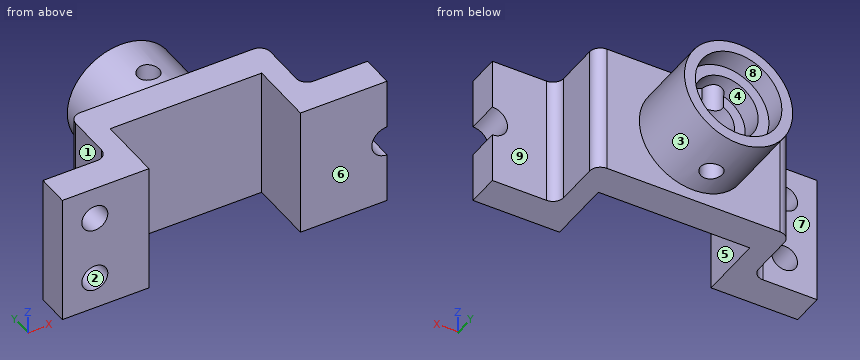
from build123d import *

# Parameters (mm, degrees)
BRACKET_BODY_DEPTH    = 30
FOOT_SLOT_A_REACH     = 88.168
FOOT_SLOT_A_SKETCH_R  = 6
FOOT_SLOT_B_REACH     = 88.168
BEARING_BOSS_SKETCH_R = 25
BEARING_BOSS_DEPTH    = 35
BORE_STEP_1_SKETCH_R  = 20
BORE_STEP_1_DEPTH     = 10
BORE_STEP_2_SKETCH_R  = 15
BORE_STEP_2_DEPTH     = 10
BORE_STEP_3_SKETCH_R  = 10
BORE_STEP_3_DEPTH     = 10
BORE_STEP_4_SKETCH_R  = 5
BORE_STEP_4_DEPTH     = 10
CROSS_HOLE_SKETCH_R   = 5
CROSS_HOLE_DEPTH      = 109.282039139
BEND_FILLET_R5_A_R    = 5
BEND_FILLET_R5_B_R    = 5
BEND_FILLET_R5_C_R    = 5


with BuildPart() as part:
    # Bracket Profile Sketch → Bracket Body (new, symmetric)
    with BuildSketch(Plane.XY):
        Polygon((-75, -30), (-35, -30), (-35, 0), (35, 0), (35, -30), (75, -30), (75, -15), (45, -15), (45, 15), (-45, 15), (-45, -15), (-75, -15), align=None)
    extrude(amount=BRACKET_BODY_DEPTH, both=True)

    # Foot Slot A Sketch → Foot Slot A (cut, up to next)
    with BuildSketch(Plane(origin=(0, -15, 0), x_dir=(1, 0, 0), z_dir=(0, 1, 0)), mode=Mode.PRIVATE) as foot_slot_a_sk1:
        with Locations(Location((-60, 15, 0), (0, 0, 180))):
            Circle(FOOT_SLOT_A_SKETCH_R)
    foot_slot_a_tool1 = extrude(foot_slot_a_sk1.sketch, amount=-FOOT_SLOT_A_REACH, mode=Mode.PRIVATE) & part.part
    # Foot Slot A Sketch → Foot Slot A (cut, up to next)
    with BuildSketch(Plane(origin=(0, -15, 0), x_dir=(1, 0, 0), z_dir=(0, 1, 0)), mode=Mode.PRIVATE) as foot_slot_a_sk2:
        with Locations(Location((-60, -15, 0), (0, 0, 180))):
            Circle(FOOT_SLOT_A_SKETCH_R)
    foot_slot_a_tool2 = extrude(foot_slot_a_sk2.sketch, amount=-FOOT_SLOT_A_REACH, mode=Mode.PRIVATE) & part.part
    add(foot_slot_a_tool1.solids().sort_by_distance((-60, -15, -15))[0], mode=Mode.SUBTRACT)
    add(foot_slot_a_tool2.solids().sort_by_distance((-60, -15, 15))[0], mode=Mode.SUBTRACT)

    # Foot Slot B Sketch → Foot Slot B (cut, up to next)
    with BuildSketch(Plane(origin=(0, -15, 0), x_dir=(1, 0, 0), z_dir=(0, 1, 0)), mode=Mode.PRIVATE) as foot_slot_b_sk1:
        with BuildLine():
            Line((75, 7), (75, -7))
            ThreePointArc((75, -7), (68, 0), (75, 7))
        make_face()
    foot_slot_b_tool1 = extrude(foot_slot_b_sk1.sketch, amount=-FOOT_SLOT_B_REACH, mode=Mode.PRIVATE) & part.part
    add(foot_slot_b_tool1.solids().sort_by_distance((72.029108, -15, 0))[0], mode=Mode.SUBTRACT)

    # Bearing Boss Sketch → Bearing Boss (add)
    with BuildSketch(Plane(origin=(0, 15, 0), x_dir=(1, 0, 0), z_dir=(0, 1, 0))):
        with Locations(Location((0, 0, 0), (0, 0, 180))):
            Circle(BEARING_BOSS_SKETCH_R)
    extrude(amount=BEARING_BOSS_DEPTH)

    # Bore Step 1 Sketch → Bore Step 1 (cut)
    with BuildSketch(Plane(origin=(0, 50, 0), x_dir=(1, 0, 0), z_dir=(0, 1, 0))):
        with Locations(Location((0, 0, 0), (0, 0, 180))):
            Circle(BORE_STEP_1_SKETCH_R)
    extrude(amount=-BORE_STEP_1_DEPTH, mode=Mode.SUBTRACT)

    # Bore Step 2 Sketch → Bore Step 2 (cut)
    with BuildSketch(Plane(origin=(0, 40, 0), x_dir=(1, 0, 0), z_dir=(0, 1, 0))):
        with Locations(Location((0, 0, 0), (0, 0, 180))):
            Circle(BORE_STEP_2_SKETCH_R)
    extrude(amount=-BORE_STEP_2_DEPTH, mode=Mode.SUBTRACT)

    # Bore Step 3 Sketch → Bore Step 3 (cut)
    with BuildSketch(Plane(origin=(0, 30, 0), x_dir=(1, 0, 0), z_dir=(0, 1, 0))):
        with Locations(Location((0, 0, 0), (0, 0, 180))):
            Circle(BORE_STEP_3_SKETCH_R)
    extrude(amount=-BORE_STEP_3_DEPTH, mode=Mode.SUBTRACT)

    # Bore Step 4 Sketch → Bore Step 4 (cut)
    with BuildSketch(Plane(origin=(0, 20, 0), x_dir=(1, 0, 0), z_dir=(0, 1, 0))):
        with Locations(Location((0, 0, 0), (0, 0, 180))):
            Circle(BORE_STEP_4_SKETCH_R)
    extrude(amount=-BORE_STEP_4_DEPTH, mode=Mode.SUBTRACT)

    # Cross Hole Sketch → Cross Hole (cut, through all)
    with BuildSketch(Plane.XY.offset(30)):
        with Locations((0, 29)):
            Circle(CROSS_HOLE_SKETCH_R)
    extrude(amount=-CROSS_HOLE_DEPTH, mode=Mode.SUBTRACT)

    # Bend Fillet R5 A
    bend_fillet_r5_a_edges = [part.edges().sort_by_distance(p)[0] for p in [
        (45, -15, 0),
    ]]
    fillet(bend_fillet_r5_a_edges, radius=BEND_FILLET_R5_A_R)

    # Bend Fillet R5 B
    bend_fillet_r5_b_edges = [part.edges().sort_by_distance(p)[0] for p in [
        (-45, 15, 0),
        (45, 15, 0),
    ]]
    fillet(bend_fillet_r5_b_edges, radius=BEND_FILLET_R5_B_R)

    # Bend Fillet R5 C
    bend_fillet_r5_c_edges = [part.edges().sort_by_distance(p)[0] for p in [
        (-45, -15, 0),
    ]]
    fillet(bend_fillet_r5_c_edges, radius=BEND_FILLET_R5_C_R)


solid = part.part
Design review of the part built by this model. Coordinates are the model's own, in mm. Face numbers are marked on the shaded views. A direction names the side the tool comes from. Round coordinates to 2 decimals unless told otherwise and drop trailing zeros. Order: outer loops, then holes, each group sorted by start corner. A loop starts at its lowest first (then second) coordinate and runs counter-clockwise, first axis right, second up. Notation, with made-up numbers: M -13.5,32 L 17.5,32 A16 ccw 17.5,48 Z; hole C -17.75,-1 d8. An arc over 180 degrees is marked long. Answer as CSV lines item,"result". Start each with the question number.
1) For pin 1 Ø3 at (x, z) = (-11, -6.5) entering from +Y; pin 2 Ø12.5 at (x, z) = (-56.5, 13.5) entering from +Y; pin 3 Ø22 at (y, z) = (4, 8.5) entering from +X; pin 4 Ø11 at (x, z) = (-60, -15) entering from -Y, all flat-tipped, find the tip position at first contact; note any pin that passes through.
2) Tool access review of the marked faces 5, 6, 7, 8 and 9: name each direction out of +Z, -Z, +X, -X, +Y, -Y from which nothing blocks a thin tool from reaching the whole face with its end or side.
3) Add section B-B (y = -3). Give the boundary of the cut face in (x, z), then the cut area to 3 significant figures.
4) Wall thickness on line 1 along Z through (x, y) = (-60, -26.75); line 2 along X through (y, z) = (-6.5, 2.5); line 3 along X through (y, z) = (2, 25): over which ranges is each line inside the solid? List them lowest first. Write a range as [from, to].
5) The part is to be moulded in two halves that separate along X. For the marked faces 1, 2, 3 and 4, say which applies: +X half, -X half, draft (parallel to the pull), parting line (faces both ways), or undercut.
6) Add section C-C (x = 0). Give the boundary of the cut face in (y, z).
7) Add section A-A (x = -60). Give the boundary of the cut face in (y, z).
8) Add section D-D (y = 36.5). Give the boundary of the cut face in (x, z).
Resolved:
1,pin 1,"y = 30"
1,pin 2,"y = -15"
1,pin 3,"x = 45"
1,pin 4,"through"
2,face 5,"+Z, -Z, -Y"
2,face 6,"+Z, -Z, +X, -X, -Y"
2,face 7,"+Z, -Z, -X, +Y"
2,face 8,"+Y"
2,face 9,"+Z, -Z, +X, +Y"
3,outline,"M -45,-30 L -35,-30 L -35,30 L -45,30 Z; M 35,-30 L 45,-30 L 45,30 L 35,30 Z"
3,area,"1,200 mm^2"
4,line 1,"[-30, -21], [-9, 9], [21, 30]"
4,line 2,"[-45, -35], [35, 45]"
4,line 3,"[-45, 45]"
5,face 1,"-X half"
5,face 2,"undercut"
5,face 3,"parting line"
5,face 4,"undercut"
6,outline,"M 0,-30 L 15,-30 L 15,-25 L 24,-25 L 24,-10 L 20,-10 L 20,-5 L 10,-5 L 10,5 L 20,5 L 20,10 L 24,10 L 24,25 L 15,25 L 15,30 L 0,30 Z; M 34,-25 L 50,-25 L 50,-20 L 40,-20 L 40,-15 L 34,-15 Z; M 34,15 L 40,15 L 40,20 L 50,20 L 50,25 L 34,25 Z"
7,outline,"M -30,-30 L -15,-30 L -15,-21 L -30,-21 Z; M -30,-9 L -15,-9 L -15,9 L -30,9 Z; M -30,21 L -15,21 L -15,30 L -30,30 Z"
8,outline,"C 0,0 d50; hole C 0,0 d30"
